For this review, take the finished solid that the model builds, in its own axes (mm). A direction names the side the tool comes from. Round coordinates to 2 decimals unless told otherwise and drop trailing zeros. Write each loop counter-clockwise with the first axis right and the second up, starting at its lowest first coordinate (ties: lowest second). Pieces come first, ordered by that corner, then holes. Notation, with made-up numbers: M -20,58.5 L 25,58.5 A34 cw 25,95.5 Z; hole C 87,-25.5 d7. An arc over 180 degrees is marked long. Answer in a Markdown table with one row per item.
```python
from build123d import *

# Parameters (mm, degrees)
BASE_BOSS_RING_SKETCH_R    = 20
BASE_BOSS_RING_SKETCH_R_2  = 10
BASE_BOSS_RING_40_DEPTH    = 20
BASE_PLATE_DEPTH           = 16
UPPER_BOSS_RING_SKETCH_R   = 33.258405
UPPER_BOSS_RING_SKETCH_R_2 = 21.112311
UPPER_BOSS_RING_DEPTH      = 10
UPRIGHT_WEB_DEPTH          = 10
MIDDLE_BOSS_SKETCH_R       = 20
MIDDLE_BOSS_SKETCH_R_2     = 10
MIDDLE_BOSS_DEPTH          = 12.5
GUSSET_RIB_DEPTH           = 6
MIDDLE_BOSS_BORE_SKETCH_R  = 10
MIDDLE_BOSS_BORE_DEPTH     = 220.228585


with BuildPart() as part:
    # Base Boss Ring Sketch → Base Boss Ring Ø40 (new body)
    with BuildSketch(Plane(origin=(0, 0, 0), x_dir=(1, 0, 0), z_dir=(0, 1, 0))):
        with Locations(Location((0, 0, 0), (0, 0, 270))):
            Circle(BASE_BOSS_RING_SKETCH_R)
        with Locations(Location((0, 0, 0), (0, 0, 270))):
            Circle(BASE_BOSS_RING_SKETCH_R_2, mode=Mode.SUBTRACT)
    extrude(amount=BASE_BOSS_RING_40_DEPTH)

    # Base Plate Sketch → Base Plate (add)
    with BuildSketch(Plane(origin=(0, 0, 0), x_dir=(1, 0, 0), z_dir=(0, 1, 0))):
        with BuildLine():
            Line((120, 60), (130, 60))
            Line((130, 60), (130, -60))
            Line((130, -60), (120, -60))
            Line((120, -60), (0, -20))
            ThreePointArc((0, -20), (20, 0), (0, 20))
            Line((0, 20), (120, 60))
        make_face()
    extrude(amount=BASE_PLATE_DEPTH)



with BuildPart() as body_2:
    # Upper Boss Ring Sketch → Upper Boss Ring (new, symmetric)
    with BuildSketch(Plane(origin=(130, 0, 0), x_dir=(0, 0, -1), z_dir=(1, 0, 0))):
        with Locations((0, 122)):
            Circle(UPPER_BOSS_RING_SKETCH_R)
        with Locations((0, 122)):
            Circle(UPPER_BOSS_RING_SKETCH_R_2, mode=Mode.SUBTRACT)
    extrude(amount=UPPER_BOSS_RING_DEPTH, both=True)


with BuildPart() as part_1:
    add(part.part)

    add(body_2.part)  # Upright Web merges body 2
    # Upright Web Sketch → Upright Web (add)
    with BuildSketch(Plane(origin=(130, 0, 0), x_dir=(0, 0, -1), z_dir=(1, 0, 0))):
        with BuildLine():
            ThreePointArc((-33.258405, 122), (0, 88.741595), (33.258405, 122))
            Line((33.258405, 122), (60, 16))
            Line((60, 16), (-60, 16))
            Line((-60, 16), (-33.258405, 122))
        make_face()
    extrude(amount=-UPRIGHT_WEB_DEPTH)



with BuildPart() as body_2_2:
    # Middle Boss Sketch → Middle Boss (new, symmetric)
    with BuildSketch(Plane.XY):
        with Locations((66.07, 56)):
            Circle(MIDDLE_BOSS_SKETCH_R)
        with Locations((66.07, 56)):
            Circle(MIDDLE_BOSS_SKETCH_R_2, mode=Mode.SUBTRACT)
    extrude(amount=MIDDLE_BOSS_DEPTH, both=True)


with BuildPart() as part_2:
    add(part_1.part)

    add(body_2_2.part)  # Gusset Rib merges body 2 2
    # Gusset Rib Sketch → Gusset Rib (add, symmetric)
    with BuildSketch(Plane.XY):
        with BuildLine():
            Line((66.07, 76), (120, 76))
            Line((120, 76), (120, 16))
            Line((120, 16), (20, 16))
            Line((20, 16), (46.07, 56))
            ThreePointArc((46.07, 56), (51.927864, 70.142136), (66.07, 76))
        make_face()
    extrude(amount=GUSSET_RIB_DEPTH, both=True)

    # Middle Boss Bore Sketch → Middle Boss Bore (cut, through all)
    with BuildSketch(Plane.XY.offset(6)):
        with Locations((66.07, 56)):
            Circle(MIDDLE_BOSS_BORE_SKETCH_R)
    extrude(amount=-MIDDLE_BOSS_BORE_DEPTH, mode=Mode.SUBTRACT)


solid = part_2.part
```
Q1. Take a section at B-B (y = 98.5). State the section outline as (x, z) points.
Found:
| item | result |
|---|---|
| outline | M 120,-39.19 L 130,-39.19 L 130,-23.53 L 140,-23.53 L 140,23.53 L 130,23.53 L 130,39.19 L 120,39.19 Z |
Q2. For probe 1 along Y at (x, z) = (66, -7); probe 2 along Y at (x, z) = (66.07, 3); probe 3 along Y at (x, z) = (133.5, 0), list the stretches that pass through material, from the lowest coordinate up.
Found:
| item | result |
|---|---|
| probe 1 | 0 to 16, 36 to 46, 66 to 76 |
| probe 2 | 0 to 46, 66 to 76 |
| probe 3 | 88.74 to 100.89, 143.11 to 155.26 |
Q3. Mouldability with a two-part tool opening along X and no side actions: class faces 4 (the face through (82, 40, 6)), 5 (the face through (74, 16, 23)), 6 (the face through (59.16, 7.89, -39.72)), 7 (the face through (125.07, 68.258, 46.816)) as +X half, -X half, draft (parallel to the pull), parting line (faces both ways), or undercut.
Found:
| item | result |
|---|---|
| face 4 | undercut |
| face 5 | undercut |
| face 6 | -X half |
| face 7 | draft |
Q4. Take a section at C-C (z = 50.5). State the section outline as (x, y) points.
Found:
| item | result |
|---|---|
| outline | M 91.5,0 L 130,0 L 130,53.66 L 120,53.66 L 120,16 L 91.5,16 Z |
Q5. Take a section at A-A (x = 110). State the section outline as (y, z) points, then the cut area to 3 significant figures.
Found:
| item | result |
|---|---|
| outline | M 0,-56.67 L 16,-56.67 L 16,-6 L 76,-6 L 76,6 L 16,6 L 16,56.67 L 0,56.67 Z |
| area | 2,530 mm² |
Q6. Take a section at D-D (z = -51). State the section outline as (x, y) points.
Found:
| item | result |
|---|---|
| outline | M 93,0 L 130,0 L 130,51.67 L 120,51.67 L 120,16 L 93,16 Z |
Q7. Machinability: for faces 1 (the face through (82, 40, -6)), 2 (the face through (132.362, 154.975, 4.33)), 3 (the face through (9, 20, -5)), which of the approach directions +Z, -Z, +X, -X, +Y, -Y give a long, thin tool a straight path to every point of the face, cutting with its end or side? Answer none if there is none.
Found:
| item | result |
|---|---|
| face 1 | -Z |
| face 2 | +X |
| face 3 | +Z, -Z, -X, +Y |
Q8. Insertion check: P1, Ø18, axis at x = 47.5, y = 56.5, coming from the +Z side; P2, Ø3.5, axis at x = 105.5, z = 1, coming from the +Y side; P3, Ø18, axis at x = 52.5, z = -38.5, coming from the +Y side. Each pin has a flat end and moves straight along its axis. Give the tip position at first contact, or say it passes through.
Found:
| item | result |
|---|---|
| P1 | z = 12.5 |
| P2 | y = 76 |
| P3 | y = 16 |
